Input: part model. Units: mm. Frame: model coordinates. Give positions to 0.01 mm unless a question says otherwise; leave off trailing zeros. Loops run counter-clockwise (first coordinate to the right, second up) from the corner with the lowest first, then second, coordinate; pieces in that order, holes last. Notation, with made-up numbers: (-1.75, -16.75) -> (55.25, -16.75) arc R34 cw to (55.25, 19.25) -> close; hole circle Ø10 at (-33, -6.75). An arc over 180 degrees is marked (long way). One line per question, with ' | ' between items.
from build123d import *

# Parameters (mm, degrees)
BOSS_EXTRUDE1_DEPTH = 5
CHAMFER1_SIZE       = 25


with BuildPart() as part:
    # Sketch1 → Boss-Extrude1 (new, symmetric)
    with BuildSketch(Plane.XY):
        Polygon((0, -280), (0, 280), (-150, 380), (-150, 400), (100, 400), (100, -400), (-150, -400), (-150, -380), align=None)
    extrude(amount=BOSS_EXTRUDE1_DEPTH, both=True)

    # Chamfer1
    chamfer1_edges = [part.edges().sort_by_distance(p)[0] for p in [
        (100, 400, 0),
        (100, -400, 0),
    ]]
    chamfer(chamfer1_edges, length=CHAMFER1_SIZE)


solid = part.part
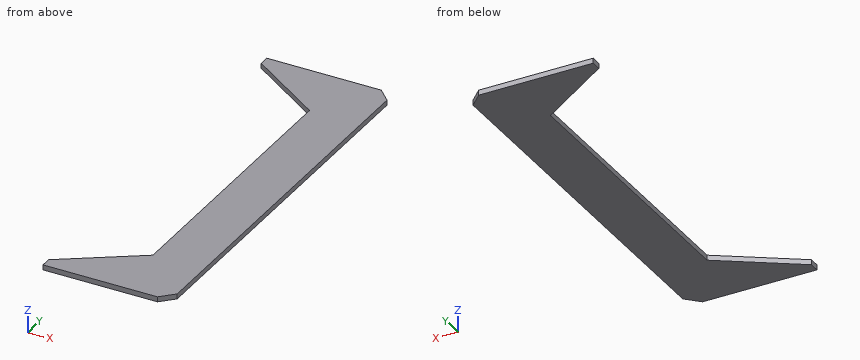
1. Section query A-A (x = -100.5). Output: boundary loops of the cut face in (y, z), then the cut area to 3 significant figures.
Determined:
outline: (-400, -5) -> (-347, -5) -> (-347, 5) -> (-400, 5) -> close; (347, -5) -> (400, -5) -> (400, 5) -> (347, 5) -> close | area: 1,060 mm2
2. Section query C-C (y = 332). Output: boundary loops of the cut face in (x, z).
Determined:
outline: (-78, -5) -> (100, -5) -> (100, 5) -> (-78, 5) -> close
3. Section query B-B (z = 1.75). Output: boundary loops of the cut face in (x, y), then the cut area to 3 significant figures.
Determined:
outline: (-150, -400) -> (75, -400) -> (100, -375) -> (100, 375) -> (75, 400) -> (-150, 400) -> (-150, 380) -> (0, 280) -> (0, -280) -> (-150, -380) -> close | area: 100,000 mm2
4. Ray query, line 1 along X through (y, z) = (189, 3); line 2 along Y through (x, z) = (-39, 4.75); line 3 along Y through (x, z) = (-63.5, 3.25). Return the intervals inside material, ascending. Write a range as from..to.
Determined:
line 1: x = 0..100 | line 2: y = -400..-306, 306..400 | line 3: y = -400..-322.33, 322.33..400
5. Section query D-D (x = -8). Output: boundary loops of the cut face in (y, z).
Determined:
outline: (-400, -5) -> (-285.33, -5) -> (-285.33, 5) -> (-400, 5) -> close; (285.33, -5) -> (400, -5) -> (400, 5) -> (285.33, 5) -> close
